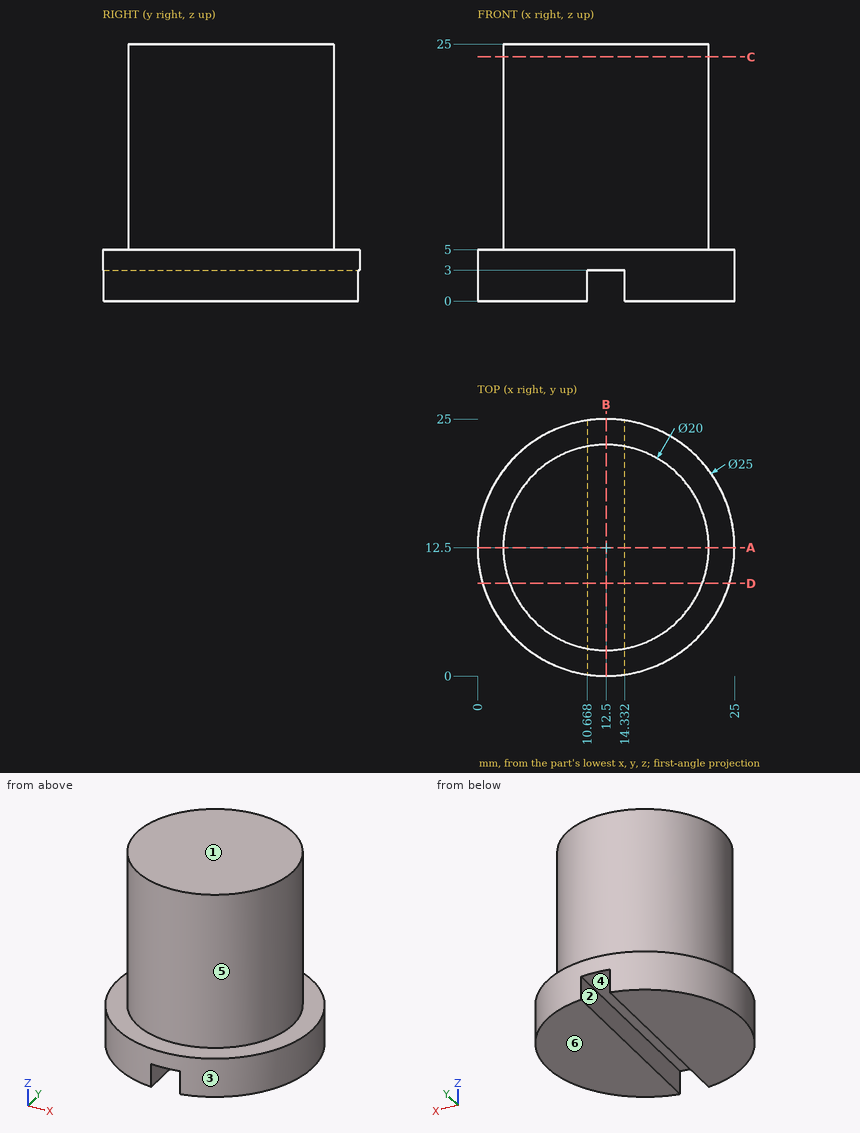
Source: three-view drawing plus pictorial views. Frame: mm from the lowest corner of the part. A direction names the side the tool comes from. Coordinates: 2 decimals unless noted, no trailing zeros. Loops run counter-clockwise (first coordinate to the right, second up) from the corner with the lowest first, then second, coordinate; pieces in that order, holes last. Notation, with made-up numbers: (39.25, -7) -> (93.25, -7) arc R14 cw to (93.25, 11) -> close; hole circle Ø7 at (61.5, 58). An arc over 180 degrees is marked (long way). Write each question's results on one line, items separated by ' | '. Start each with the question number.
Q1. Section B-B, the plane x = 12.5. Return the cut outline in (y, z), plus the area to 3 significant figures.
Q2. Section C-C, the plane z = 23.75. Return the cut outline in (x, y), plus the area to 3 significant figures.
Q3. Pin query (flat end, axial travel): pin 1 (2 mm diameter, centred on x = 17, y = 19.5, fed in from -Z); pin 2 (1.8 mm diameter, centred on x = 12, y = 17.5, fed in from -Z); pin 3 (1.5 mm diameter, centred on y = 8.5, z = 1.5, fed in from -X); pin 4 (1 mm diameter, centred on x = 9, z = 21.5, fed in from -Y). Return the tip coordinate at first contact, or that it passes through.
Q4. Pull-direction query (X, two-part tool) for the marked faces 1, 2, 3 and 4; classes: released by +X, released by -X, zero draft, split by the parting line, or undercut.
Q5. Ray query, line 1 (Z direction, x = 24, y = 14); line 2 (Z direction, x = 13, y = 6); line 3 (Y direction, x = 12.75, z = 15.25). Return the intervals inside material, ascending. Write a range as from..to.
Q6. Section A-A, the plane y = 12.5. Return the cut outline in (x, z).
Q7. Reachability of the marked faces 5 and 6 from +Z, -Z, +X, -X, +Y, -Y: full face, straight path, thin tool, end or side. Return the list, or none.
Q8. Section D-D, the plane y = 9. Return the cut outline in (x, z).
Found:
1) outline: (0, 3) -> (25, 3) -> (25, 5) -> (22.5, 5) -> (22.5, 25) -> (2.5, 25) -> (2.5, 5) -> (0, 5) -> close | area: 450 mm2
2) outline: circle Ø20 at (12.5, 12.5) | area: 314 mm2
3) pin 1: z = 0 | pin 2: z = 3 | pin 3: x = 0.43 | pin 4: y = 2.96
4) face 1: zero draft | face 2: undercut | face 3: split by the parting line | face 4: undercut
5) line 1: 0..5 | line 2: 3..25 | line 3: 2.5..22.5
6) outline: (0, 0) -> (10.67, 0) -> (10.67, 3) -> (14.33, 3) -> (14.33, 0) -> (25, 0) -> (25, 5) -> (22.5, 5) -> (22.5, 25) -> (2.5, 25) -> (2.5, 5) -> (0, 5) -> close
7) face 5: +Z | face 6: -Z, +X, -X, +Y, -Y
8) outline: (0.5, 0) -> (10.67, 0) -> (10.67, 3) -> (14.33, 3) -> (14.33, 0) -> (24.5, 0) -> (24.5, 5) -> (21.87, 5) -> (21.87, 25) -> (3.13, 25) -> (3.13, 5) -> (0.5, 5) -> close
